For this review, take the finished solid that the model builds, in its own axes (mm). A direction names the side the tool comes from. Give positions to 0.01 mm unless a question says otherwise; leave off trailing zeros. Loops run counter-clockwise (first coordinate to the right, second up) from the corner with the lowest first, then second, coordinate; pieces in that order, holes last. Notation, with made-up numbers: M 37.25,-9.75 L 60.25,-9.75 A9 cw 60.25,-5.75 Z; hole C 44.5,23.5 d8. An arc over 180 degrees is marked long. Use CSV: the item, a comma, the result in double quotes. Start each with the question number.
1. Tool access review of faces 1 (the face through (-23, -4, 40)), 2 (the face through (-30, 0, 24)): name each direction out of +Z, -Z, +X, -X, +Y, -Y from which nothing blocks a thin tool from reaching the whole face with its end or side.
2. Take a section at A-A, the plane x = -22.5. Write out the cut boundary in (y, z), and give its area (3 significant figures).
3. Take a section at D-D, the plane x = -12. Write out the cut boundary in (y, z), and give its area (3 significant figures).
4. To check wall thickness, follow line 1 (Y direction, x = -22.5, z = 42.5); line 2 (X direction, y = -2.75, z = 37); line 3 (X direction, y = -1, z = 29.5). State the ranges of each line that lie inside material, in increasing order. Write a range as [from, to].
5. Take a section at B-B, the plane y = 0. Write out the cut boundary in (x, z), and give its area (3 significant figures).
6. Insertion check: P1, Ø10, axis at x = 22.5, y = 0, coming from the +Z side. The pin has a flat end and moves straight along its axis. Give the tip position at first contact, or say it passes through.
7. Take a section at C-C, the plane z = 41.5. Write out the cut boundary in (x, y), and give its area (3 significant figures).
8. The part is to be moulded in two halves that separate along Y. For faces 3 (the face through (9.92, 0.14, 29.01)), 4 (the face through (22, -4, 40)), 5 (the face through (0, 10, 24)), say which applies: pulls with the +Y half, pulls with the -Y half, needs draft (parallel to the pull), parting line crosses it, or undercut.
from build123d import *

# Parameters (mm, degrees)
SKETCH1_W                                           = 60
SKETCH1_H                                           = 20
BOSS_EXTRUDE1_DEPTH                                 = 48
CBORE_FOR_M6_HEX_SOCKET_HEAD_CAP_SCREW1_D           = 6.6
CBORE_FOR_M6_HEX_SOCKET_HEAD_CAP_SCREW1_CBORE_D     = 11
CBORE_FOR_M6_HEX_SOCKET_HEAD_CAP_SCREW1_CBORE_DEPTH = 8
M8_TAPPED_HOLE1_D                                   = 6.8
M10X1_0_TAPPED_HOLE1_D                              = 9
CHAMFER1_SIZE                                       = 1


with BuildPart() as part:
    # Sketch1 → Boss-Extrude1 (new body)
    with BuildSketch(Plane.XY):
        Rectangle(SKETCH1_W, SKETCH1_H)
    extrude(amount=BOSS_EXTRUDE1_DEPTH)

    # CBORE for M6 Hex Socket Head Cap Screw1 (through all)
    with Locations(Plane.XY.offset(48)):
        with Locations((-22.5, 0), (22.5, 0)):
            CounterBoreHole(CBORE_FOR_M6_HEX_SOCKET_HEAD_CAP_SCREW1_D / 2, CBORE_FOR_M6_HEX_SOCKET_HEAD_CAP_SCREW1_CBORE_D / 2, CBORE_FOR_M6_HEX_SOCKET_HEAD_CAP_SCREW1_CBORE_DEPTH)

    # M8 Tapped Hole1 (through all)
    with Locations(Plane.XZ.offset(10)):
        with Locations((-12, 33)):
            Hole(M8_TAPPED_HOLE1_D / 2)

    # M10x1.0 Tapped Hole1 (through all)
    with Locations(Plane.XZ.offset(10)):
        with Locations((12, 33)):
            Hole(M10X1_0_TAPPED_HOLE1_D / 2)

    # Chamfer1
    chamfer1_edges = [part.edges().sort_by_distance(p)[0] for p in [
        (30, -10, 24),
        (-30, -10, 24),
        (-30, 10, 24),
        (30, 10, 24),
    ]]
    chamfer(chamfer1_edges, length=CHAMFER1_SIZE)


solid = part.part
Result set:
1,face 1,"+Z"
1,face 2,"+Z, -Z, -X, +Y, -Y"
2,outline,"M -10,0 L -3.3,0 L -3.3,40 L -5.5,40 L -5.5,48 L -10,48 Z; M 3.3,0 L 10,0 L 10,48 L 5.5,48 L 5.5,40 L 3.3,40 Z"
2,area,"608 mm2"
3,outline,"M -10,0 L 10,0 L 10,29.6 L -10,29.6 Z; M -10,36.4 L 10,36.4 L 10,48 L -10,48 Z"
3,area,"824 mm2"
4,line 1,"[-10, -5.5], [5.5, 10]"
4,line 2,"[-30, -24.32], [-20.68, 9.94], [14.06, 20.68], [24.32, 30]"
4,line 3,"[-30, -25.64], [-19.36, 9.17], [14.83, 19.36], [25.64, 30]"
5,outline,"M -30,0 L -25.8,0 L -25.8,40 L -28,40 L -28,48 L -30,48 Z; M -19.2,0 L 19.2,0 L 19.2,40 L 17,40 L 17,48 L -17,48 L -17,40 L -19.2,40 Z; M 25.8,0 L 30,0 L 30,48 L 28,48 L 28,40 L 25.8,40 Z; hole C -12,33 d6.8; hole C 12,33 d9"
5,area,"2,080 mm2"
6,P1,"z = 40"
7,outline,"M -30,-9 L -29,-10 L 29,-10 L 30,-9 L 30,9 L 29,10 L -29,10 L -30,9 Z; hole C -22.5,0 d11; hole C 22.5,0 d11"
7,area,"1,010 mm2"
8,face 3,"needs draft"
8,face 4,"undercut"
8,face 5,"pulls with the +Y half"
